```python
from build123d import *

# Parameters (mm, degrees)
EXTRUDE_THIN1_DEPTH = 1020


with BuildPart() as part:
    # Sketch1 → Extrude-Thin1 (new, symmetric)
    with BuildSketch(Plane(origin=(0, 0, 0), x_dir=(1, 0, 0), z_dir=(0, 1, 0))):
        with BuildLine():
            Line((-40, 25), (40, 25))
            ThreePointArc((40, 25), (47.071067812, 22.071067812), (50, 15))
            Line((50, 15), (50, -15))
            ThreePointArc((50, -15), (47.071067812, -22.071067812), (40, -25))
            Line((40, -25), (-40, -25))
            ThreePointArc((-40, -25), (-47.071067812, -22.071067812), (-50, -15))
            Line((-50, -15), (-50, 15))
            ThreePointArc((-50, 15), (-47.071067812, 22.071067812), (-40, 25))
        make_face()
        with BuildLine():
            Line((-40, 22), (40, 22))
            ThreePointArc((40, 22), (44.949747468, 19.949747468), (47, 15))
            Line((47, 15), (47, -15))
            ThreePointArc((47, -15), (44.949747468, -19.949747468), (40, -22))
            Line((40, -22), (-40, -22))
            ThreePointArc((-40, -22), (-44.949747468, -19.949747468), (-47, -15))
            Line((-47, -15), (-47, 15))
            ThreePointArc((-47, 15), (-44.949747468, 19.949747468), (-40, 22))
        make_face(mode=Mode.SUBTRACT)
    extrude(amount=EXTRUDE_THIN1_DEPTH, both=True)


solid = part.part
```
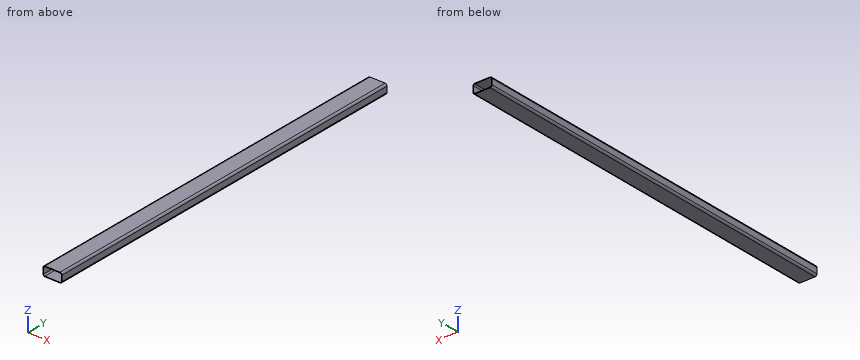
Could you check a few things on this model? Use its own coordinates, in mm. Coordinates: 2 decimals unless noted, no trailing zeros. Loops run counter-clockwise (first coordinate to the right, second up) from the corner with the lowest first, then second, coordinate; pieces in that order, holes last.
1) Imagine slicing it at A-A (z = 0). List the corners of the cut face in (x, y) for me.
Reported:
outline: (-50, -1020) - (-47, -1020) - (-47, 1020) - (-50, 1020) - close; (47, -1020) - (50, -1020) - (50, 1020) - (47, 1020) - close
2) Imagine slicing it at C-C (x = 17). List the corners of the cut face in (y, z) for me, and give its area (3 significant figures).
Reported:
outline: (-1020, -25) - (1020, -25) - (1020, -22) - (-1020, -22) - close; (-1020, 22) - (1020, 22) - (1020, 25) - (-1020, 25) - close
area: 12,200 mm2
3) Will this pin go through, and if not, where does the flat tip stop? pin 1 Ø10 at (x, z) = (-28, -16.5) entering from -Y.
Reported:
pin 1: passes through
4) Imagine slicing it at B-B (y = 431.5). List the corners of the cut face in (x, z) for me.
Reported:
outline: (-50, -15) arc R10 ccw to (-40, -25) - (40, -25) arc R10 ccw to (50, -15) - (50, 15) arc R10 ccw to (40, 25) - (-40, 25) arc R10 ccw to (-50, 15) - close; hole (-47, -15) arc R7 ccw to (-40, -22) - (40, -22) arc R7 ccw to (47, -15) - (47, 15) arc R7 ccw to (40, 22) - (-40, 22) arc R7 ccw to (-47, 15) - close
5) Please list where these lines run through material, in increasing order: line 1 along Z through (x, y) = (24, 366); line 2 along X through (y, z) = (-627, -15); line 3 along X through (y, z) = (-71.5, -16).
Reported:
line 1: z = -25 to -22, 22 to 25
line 2: x = -50 to -47, 47 to 50
line 3: x = -49.95 to -46.93, 46.93 to 49.95
